The model under review builds one solid part; all positions refer to its coordinate system, in mm. A direction names the side the tool comes from. Round coordinates to 2 decimals unless told otherwise and drop trailing zeros. Order: outer loops, then holes, each group sorted by start corner. A loop starts at its lowest first (then second) coordinate and runs counter-clockwise, first axis right, second up. Notation, with made-up numbers: M -4,59.25 L 17,59.25 A24 ccw 17,90.25 Z; hole C -25.5,10.5 d2. An arc over 180 degrees is marked long. Use a Markdown table: item, result. Add a question column.
1. Consider section A-A on x = 22.5. State the section outline as (y, z) points.
2. To check wall thickness, follow probe 1 along X at (y, z) = (3.5, 1.25); probe 2 along Y at (x, z) = (13, -0.25); probe 3 along Z at (x, y) = (10, 2). State the ranges of each line that lie inside material, in increasing order.
3. Consider section B-B on y = 5. State the section outline as (x, z) points (3 decimals).
4. For faces 1 (the cylindrical face through (19.288, 3.905, -0.867)), 2 (the flat face through (31, 0, 0)), 3 (the flat face through (2.129, -0.008, 2.417)), list the 3-axis set-ups (+Z, -Z, +X, -X, +Y, -Y) from which the entire face can be reached by the end or side of a thin tool; tool diameter is ignored.
5. Insertion check: P1, Ø5, axis at x = 10.5, y = -2.5, coming from the +Z side; P2, Ø4, axis at x = 25, y = 0.5, coming from the -Z side; P3, Ø3, axis at x = 26.5, z = 4, coming from the -Y side. Each pin has a flat end and moves straight along its axis. Give the tip position at first contact, or say it passes through.
6. The part is to be moulded in two halves that separate along X. For faces 4 (the cylindrical face through (4.35, 7.81, -1.73)), 5 (the flat face through (6, 3.4, -3.4)), 6 (the flat face through (1.775, -0.384, 1.49)), 7 (the cylindrical face through (7.544, -1.04, 3.304)), say which applies: +X half, -X half, draft (parallel to the pull), parting line (faces both ways), or undercut.
from build123d import *


with BuildPart() as part:
    # 草图2 → Revolve 709 (revolve)
    with BuildSketch(Plane.XY, mode=Mode.PRIVATE) as revolve_709_sk:
        with BuildLine():
            Line((0, 0), (31, 0))
            Line((31, 0), (31, 4))
            Line((31, 4), (8.5, 4))
            Line((8.5, 4), (7.964, 3.464))
            Line((7.964, 3.464), (7.136, 3.464))
            ThreePointArc((7.136, 3.464), (6.332726697, 3.796726697), (6, 4.6))
            Line((6, 4.6), (6, 8))
            Line((6, 8), (2.753049234, 8))
            ThreePointArc((2.753049234, 8), (0.707515305, 4.230226947), (0, 0))
        make_face()
    revolve(revolve_709_sk.sketch.rotate(Axis((-1.331757704, 0, 0), (1, 0, 0)), 90), axis=Axis((-1.331757704, 0, 0), (1, 0, 0)))

    # 草图3 → 切除-旋转1 (revolve, cut)
    with BuildSketch(Plane.XY, mode=Mode.PRIVATE) as cut_revolve_1_sk:
        Polygon((30.381770007, 4), (31.631770007, 4), (31, 2.9175), align=None)
    revolve(cut_revolve_1_sk.sketch.rotate(Axis((-0.242766179, 0, 0), (1, 0, 0)), 90), axis=Axis((-0.242766179, 0, 0), (1, 0, 0)), mode=Mode.SUBTRACT)

    # 草图5 → 切除-放样1 section 0
    with BuildSketch(Plane(origin=(0, 0, 0), x_dir=(0, 0, -1), z_dir=(1, 0, 0)), mode=Mode.PRIVATE) as loft_1_s0:
        with BuildLine():
            Line((0.625, 4.5), (-0.625, 4.5))
            Line((-0.625, 4.5), (-0.625, -4.5))
            Line((-0.625, -4.5), (0.625, -4.5))
            Line((0.625, -4.5), (0.625, 4.5))
        make_face()
    loft_1 = loft([Vertex(4.6, 0, 0), loft_1_s0.sketch], mode=Mode.SUBTRACT)

    # 镜向1: 切除-放样1 across plane
    add(loft_1.mirror(Plane(origin=(0, 0, 0), x_dir=(0, 0.7071067811865462, 0.7071067811865488), z_dir=(0, -0.7071067811865488, 0.7071067811865462))), mode=Mode.SUBTRACT)


solid = part.part
Answer block:
| question | item | result |
|---|---|---|
| 1 | outline | C 0,0 d8 |
| 2 | probe 1 | 0.54 to 6.42, 8.22 to 30.54 |
| 2 | probe 2 | -3.99 to 3.99 |
| 2 | probe 3 | -3.46 to 3.46 |
| 3 | outline | M 2.753,-6.245 L 6,-6.245 L 6,6.245 L 2.753,6.245 A12 ccw Z |
| 4 | face 1 | +X |
| 4 | face 2 | +Z, -Z, +X, +Y, -Y |
| 4 | face 3 | -X |
| 5 | P1 | z = 4 |
| 5 | P2 | z = -4 |
| 5 | P3 | y = -3.12 |
| 6 | face 4 | draft |
| 6 | face 5 | +X half |
| 6 | face 6 | -X half |
| 6 | face 7 | undercut |
